Can you work these out from the model? Positions are in its coordinate system, mm. Give positions to 0.01 mm unless a question says otherwise; leave off trailing zeros. Return JSON: item names as keys, results as strings. Group by question number.
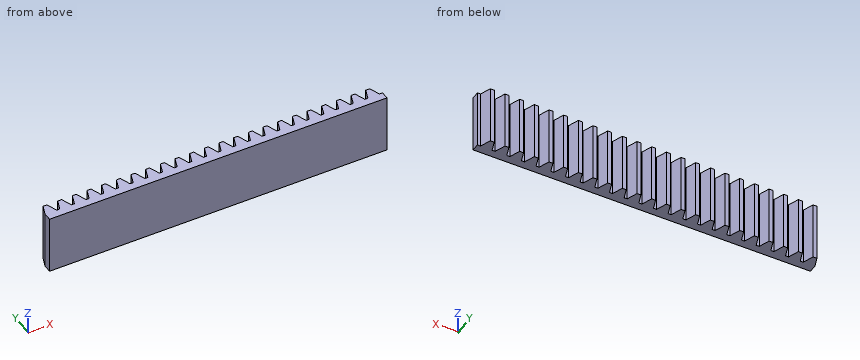
from build123d import *

# Parameters (mm, degrees)
SKETCH1_W           = 5
SKETCH1_H           = 5
BOSS_EXTRUDE1_DEPTH = 150
BOSS_EXTRUDE2_DEPTH = 150


with BuildPart() as part:
    # Sketch1 → Boss-Extrude1 (new body)
    with BuildSketch(Plane.XY):
        with Locations((2.5, 2.5)):
            Rectangle(SKETCH1_W, SKETCH1_H)
    extrude(amount=BOSS_EXTRUDE1_DEPTH)

    # Sketch2 → Boss-Extrude2 (add)
    with BuildSketch(Plane.XY):
        Polygon((0, 20), (9.827196325, 47), (19.941466624, 47), (29.76866295, 20), (37.699111843, 20), (47.526308168, 47), (57.640578467, 47), (67.467774793, 20), (75.398223686, 20), (85.225420011, 47), (95.33969031, 47), (105.166886636, 20), (113.097335529, 20), (122.924531854, 47), (133.038802154, 47), (142.865998479, 20), (150.796447372, 20), (160.623643697, 47), (170.737913997, 47), (180.565110322, 20), (188.495559215, 20), (198.322755541, 47), (208.43702584, 47), (218.264222165, 20), (226.194671058, 20), (236.021867384, 47), (246.136137683, 47), (255.963334008, 20), (263.893782902, 20), (273.720979227, 47), (283.835249526, 47), (293.662445851, 20), (301.592894745, 20), (311.42009107, 47), (321.534361369, 47), (331.361557694, 20), (339.292006588, 20), (349.119202913, 47), (359.233473212, 47), (369.060669537, 20), (376.991118431, 20), (386.818314756, 47), (396.932585055, 47), (406.75978138, 20), (414.690230274, 20), (424.517426599, 47), (434.631696898, 47), (444.458893223, 20), (452.389342117, 20), (462.216538442, 47), (472.330808741, 47), (482.158005066, 20), (490.08845396, 20), (499.915650285, 47), (510.029920584, 47), (519.85711691, 20), (527.787565803, 20), (537.614762128, 47), (547.729032427, 47), (557.556228753, 20), (565.486677646, 20), (575.313873971, 47), (585.42814427, 47), (595.255340596, 20), (603.185789489, 20), (613.012985814, 47), (623.127256114, 47), (632.954452439, 20), (640.884901332, 20), (650.712097658, 47), (660.826367957, 47), (670.653564282, 20), (678.584013175, 20), (688.411209501, 47), (698.5254798, 47), (708.352676125, 20), (716.283125018, 20), (726.110321344, 47), (736.224591643, 47), (746.051787968, 20), (753.982236862, 20), (763.809433187, 47), (773.923703486, 47), (783.750899811, 20), (791.681348705, 20), (801.50854503, 47), (811.622815329, 47), (821.450011654, 20), (829.380460548, 20), (839.207656873, 47), (849.321927172, 47), (859.149123497, 20), (867.079572391, 20), (867.079572391, 0), (0, 0), align=None)
    extrude(amount=BOSS_EXTRUDE2_DEPTH)


solid = part.part
1) I need wall thicknesses on line 1 along Y through (x, z) = (822, 57). Which ranges of the line are inside material? Lowest first, please.
2) Will these pins go through, and if not, where does the flat tip stop? pin 1 Ø1 at (y, z) = (40.5, 17.5) entering from +X; pin 2 Ø2.5 at (x, z) = (297, 78.5) entering from +Y; pin 3 Ø4 at (x, y) = (492, 34.5) entering from -Z; pin 4 Ø3 at (y, z) = (26, 114) entering from -X.
3) Imagine slicing it at A-A, the plane y = 36. Count the separate pieces of the cut face and the enclosed holes in it, and give its area (3 significant figures).
Resolved:
{
 "1": {"line 1": "0 to 20"},
 "2": {"pin 1": "x = 851.87", "pin 2": "y = 20", "pin 3": "through", "pin 4": "x = 1.64"},
 "3": {"separate pieces": "23", "enclosed holes": "0", "area": "62,500 mm^2"}
}
